Check sheet for the modelled part. Datum: model origin and axes. Units: mm. Face numbers are marked on the shaded views. A direction names the side the tool comes from. Round coordinates to 2 decimals unless told otherwise and drop trailing zeros. Loops run counter-clockwise (first coordinate to the right, second up) from the corner with the lowest first, then second, coordinate; pieces in that order, holes last. Notation, with made-up numbers: (48.25, 45) - (64.25, 45) arc R20 ccw to (64.25, 72) - close; hole circle Ø10 at (25, 9). An arc over 180 degrees is marked (long way). Put each result on its own line as item: value. Start each with the question number.
Item 1: Section check C-C, the plane y = 4. Record the cut outline in (x, z), and give its area (3 significant figures).
Item 2: Draft check along X on the marked faces 1, 2 and 3. Enter one of: pulls with the +X half, pulls with the -X half, needs draft (parallel to the pull), parting line crosses it, or undercut.
Item 3: Section check B-B, the plane x = 5. Record the cut outline in (y, z), and give its area (3 significant figures).
Item 4: Section check A-A, the plane z = 4.5. Record the cut outline in (x, y).
Item 5: Material ranges on line 1 along X through (y, z) = (5.5, 4); line 2 along X through (y, z) = (12, 0.8); line 3 along Y through (x, z) = (14.25, 7.25), recorded low to high.
Item 6: Tool access check on the marked faces 4, 5 and 6. Record the directions out of +Z, -Z, +X, -X, +Y, -Y that give a thin tool (end or side, any length) a straight path to the whole face; none if there is none.
Item 7: Gauge pin test, flat ends, axial feed: pin 1 Ø2 at (y, z) = (-2, 2.5) entering from +X; pin 2 Ø1.8 at (x, z) = (3.5, 2.5) entering from +Y; pin 3 Ø2 at (y, z) = (-2, 2.5) entering from -X; pin 4 Ø1.4 at (x, y) = (5, 4) entering from +Z. Record the tip position at first contact, or that the pin passes through.
Item 8: Section check D-D, the plane z = 6.75. Record the cut outline in (x, y).
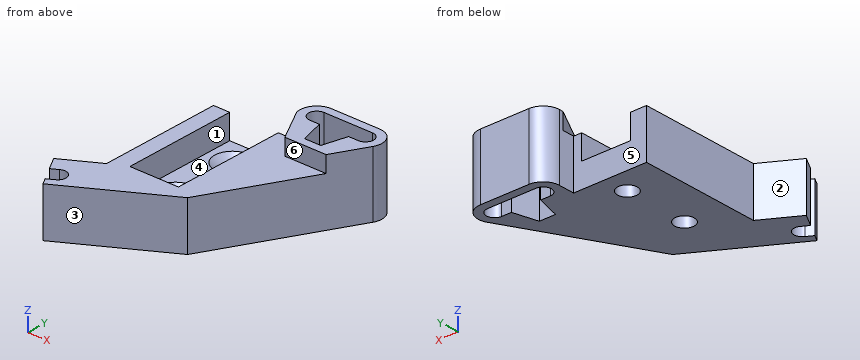
from build123d import *

# Parameters (mm, degrees)
L_BRACKET_BODY_DEPTH             = 6
TRAPEZOID_SLOT_BOSS_DEPTH        = 2
POCKET_CUT_DEPTH                 = 14
M2_COUNTERSUNK_HOLES_D           = 2.4
M2_COUNTERSUNK_HOLES_CSINK_D     = 4.4
M2_COUNTERSUNK_HOLES_CSINK_ANGLE = 90


with BuildPart() as part:
    # L Bracket Profile Sketch → L Bracket Body (new body)
    # profile 1 of 2: a face of its own
    with BuildSketch(Plane.XY):
        with BuildLine():
            Line((0, 15), (0, 0))
            Line((0, 0), (-4.330127019, -2.5))
            Line((-4.330127019, -2.5), (-3.329569645, -4.233016207))
            Line((-3.329569645, -4.233016207), (-2.504424414, -3.756618386))
            ThreePointArc((-2.504424414, -3.756618386), (-1.098076211, -4.098076211), (-1.505539161, -5.486738395))
            Line((-1.505539161, -5.486738395), (-2.330684392, -5.963136216))
            Line((-2.330684392, -5.963136216), (-1.830127019, -6.830127019))
            Line((-1.830127019, -6.830127019), (10, 0))
            Line((10, 0), (16.549529843, 12))
            Line((16.549529843, 12), (14, 12))
            Line((14, 12), (11.450470157, 12))
            Line((11.450470157, 12), (9.244459544, 16.041836283))
            ThreePointArc((9.244459544, 16.041836283), (9.062078315, 16.505571497), (9, 17))
            Line((9, 17), (9, 15))
            Line((9, 15), (0, 15))
        make_face()
    # profile 2 of 2: a face of its own
    with BuildSketch(Plane.XY):
        with BuildLine():
            ThreePointArc((11, 19), (9.585786438, 18.414213562), (9, 17))
            ThreePointArc((9, 17), (9.062078315, 16.505571497), (9.244459544, 16.041836283))
            Line((9.244459544, 16.041836283), (11.450470157, 12))
            Line((11.450470157, 12), (14, 12))
            Line((14, 12), (16.549529843, 12))
            Line((16.549529843, 12), (18.755540456, 16.041836283))
            ThreePointArc((18.755540456, 16.041836283), (18.719931312, 18.020703817), (17, 19))
            Line((17, 19), (11, 19))
        make_face()
        with BuildLine():
            Line((15, 13), (13, 13))
            Line((13, 13), (12.196152423, 16))
            Line((12.196152423, 16), (11, 16))
            ThreePointArc((11, 16), (10, 17), (11, 18))
            Line((11, 18), (17, 18))
            ThreePointArc((17, 18), (18, 17), (17, 16))
            Line((17, 16), (15.803847577, 16))
            Line((15.803847577, 16), (15, 13))
        make_face(mode=Mode.SUBTRACT)
    extrude(amount=L_BRACKET_BODY_DEPTH)

    # Trapezoid Slot Boss Sketch → Trapezoid Slot Boss (add)
    with BuildSketch(Plane.XY.offset(6)):
        with BuildLine():
            Line((14, 12), (16.549529843, 12))
            Line((16.549529843, 12), (18.755540456, 16.041836283))
            ThreePointArc((18.755540456, 16.041836283), (18.719931312, 18.020703817), (17, 19))
            Line((17, 19), (11, 19))
            ThreePointArc((11, 19), (9.585786438, 18.414213562), (9, 17))
            Line((9, 17), (9, 16.489733247))
            Line((9, 16.489733247), (11.450470157, 12))
            Line((11.450470157, 12), (14, 12))
        make_face()
        with BuildLine():
            Line((11, 18), (17, 18))
            ThreePointArc((17, 18), (18, 17), (17, 16))
            Line((17, 16), (15.803847577, 16))
            Line((15.803847577, 16), (15, 13))
            Line((15, 13), (13, 13))
            Line((13, 13), (12.196152423, 16))
            Line((12.196152423, 16), (11, 16))
            ThreePointArc((11, 16), (10, 17), (11, 18))
        make_face(mode=Mode.SUBTRACT)
    extrude(amount=TRAPEZOID_SLOT_BOSS_DEPTH)

    # Pocket Cut Sketch → Pocket Cut (cut)
    with BuildSketch(Plane(origin=(0, 15, 0), x_dir=(1, 0, 0), z_dir=(0, 1, 0))):
        Polygon((2, -3), (2, -6), (5, -6), (8, -6), (8, -3), (5, -3), align=None)
    extrude(amount=-POCKET_CUT_DEPTH, mode=Mode.SUBTRACT)

    # M2 Countersunk Holes (through all)
    with Locations(Plane.XY.offset(3)):
        with Locations((5, 12), (5, 4)):
            CounterSinkHole(M2_COUNTERSUNK_HOLES_D / 2, M2_COUNTERSUNK_HOLES_CSINK_D / 2, counter_sink_angle=M2_COUNTERSUNK_HOLES_CSINK_ANGLE)


solid = part.part
Check result:
1. outline: (0, 0) - (3.8, 0) - (3.8, 2) - (2.8, 3) - (2, 3) - (2, 6) - (0, 6) - close; (6.2, 0) - (12.18, 0) - (12.18, 6) - (8, 6) - (8, 3) - (7.2, 3) - (6.2, 2) - close
1. area: 46.9 mm²
2. face 1: undercut
2. face 2: pulls with the -X half
2. face 3: pulls with the +X half
3. outline: (-2.89, 0) - (2.8, 0) - (2.8, 2) - (1.8, 3) - (1, 3) - (1, 6) - (-2.89, 6) - close; (5.2, 0) - (10.8, 0) - (10.8, 2) - (9.8, 3) - (6.2, 3) - (5.2, 2) - close; (13.2, 0) - (15, 0) - (15, 3) - (14.2, 3) - (13.2, 2) - close
3. area: 48.9 mm²
4. outline: (-4.33, -2.5) - (-3.33, -4.23) - (-2.5, -3.76) arc R1 cw (long way) to (-1.51, -5.49) - (-2.33, -5.96) - (-1.83, -6.83) - (10, 0) - (18.76, 16.04) arc R2 ccw to (17, 19) - (11, 19) arc R2 ccw to (9, 17) - (9, 15) - (8, 15) - (8, 1) - (2, 1) - (2, 15) - (0, 15) - (0, 0) - close; hole (11, 16) - (12.2, 16) - (13, 13) - (15, 13) - (15.8, 16) - (17, 16) arc R1 ccw to (17, 18) - (11, 18) arc R1 ccw to start
5. line 1: 0 to 2, 8 to 13
5. line 2: 0 to 3.8, 6.2 to 16.55
5. line 3: 12 to 13, 18 to 19
6. face 4: +Z, +Y
6. face 5: +Z, -Z, -X, +Y
6. face 6: +Z, +X, -X, -Y
7. pin 1: x = 8.27
7. pin 2: y = 15
7. pin 3: x = -4.33
7. pin 4: through
8. outline: (9, 16.49) - (11.45, 12) - (16.55, 12) - (18.76, 16.04) arc R2 ccw to (17, 19) - (11, 19) arc R2 ccw to (9, 17) - close; hole (11, 16) - (12.2, 16) - (13, 13) - (15, 13) - (15.8, 16) - (17, 16) arc R1 ccw to (17, 18) - (11, 18) arc R1 ccw to start
